Design review of the part shown in the three views and the two pictorial views. Dimensions are in mm from the part's minimum x, y and z. A direction names the side the tool comes from. Round coordinates to 2 decimals unless told otherwise and drop trailing zeros. Loops run counter-clockwise (first coordinate to the right, second up) from the corner with the lowest first, then second, coordinate; pieces in that order, holes last. Notation, with made-up numbers: (-27, 79) -> (11, 79) arc R11 cw to (11, 100) -> close; hole circle Ø6 at (68, 50). An arc over 180 degrees is marked (long way). Use CSV: the item, a comma, the result in double quotes. Start each with the question number.
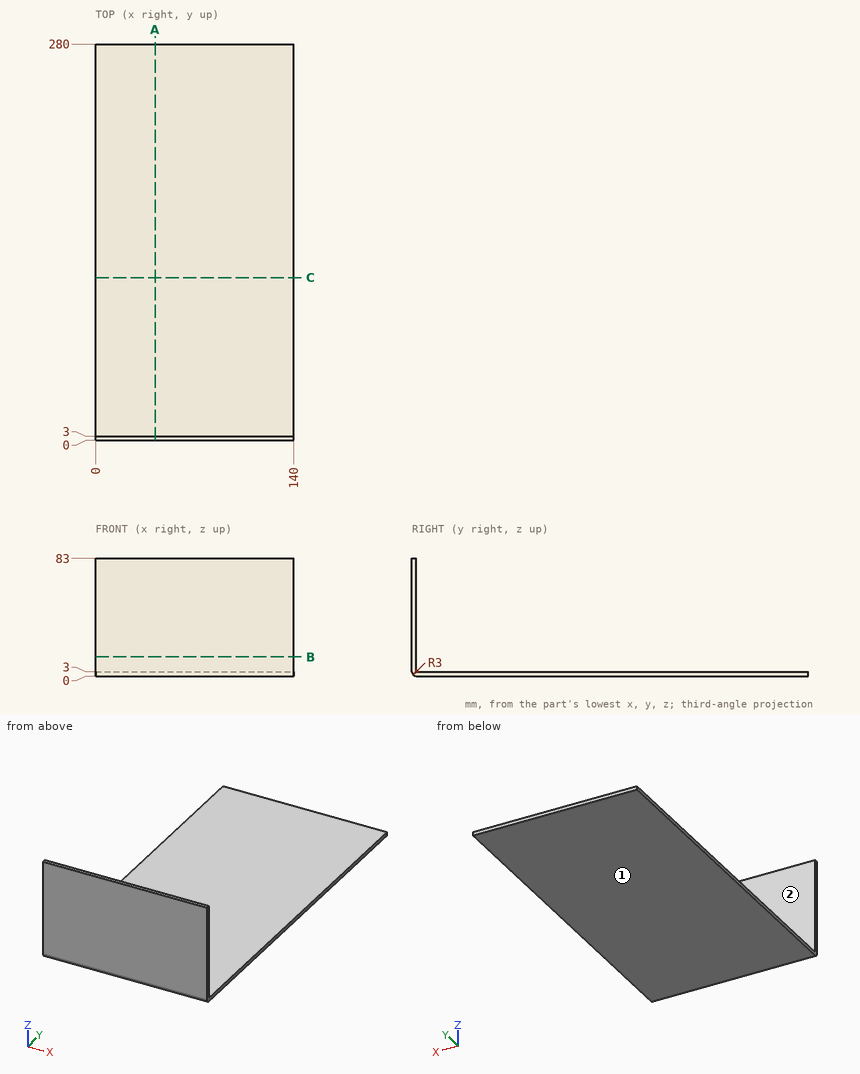
1. For the marked faces 1 and 2, list the 3-axis set-ups (+Z, -Z, +X, -X, +Y, -Y) from which the entire face can be reached by the end or side of a thin tool; tool diameter is ignored.
2. For line 1 along Z through (x, y) = (46.5, 228), list the stretches that pass through material, from the lowest coordinate up. Write a range as from..to.
3. Take a section at A-A, the plane x = 42. Give the boundary of the cut face in (y, z), then the cut area to 3 significant figures.
4. Take a section at B-B, the plane z = 13.5. Give the boundary of the cut face in (x, y).
5. Clearance check with flat-ended pins moving along their axes: P1, Ø4, axis at x = 54, z = 54, coming from the +Y side; P2, Ø8, axis at x = 93.5, y = 219, coming from the +Z side. State where each tip first meets the part, or that it passes through.
Results:
1,face 1,"-Z, +X, -X, +Y, -Y"
1,face 2,"+Z, +X, -X, +Y"
2,line 1,"0..3"
3,outline,"(0, 3) arc R3 ccw to (3, 0) -> (280, 0) -> (280, 3) -> (3, 3) -> (3, 83) -> (0, 83) -> close"
3,area,"1,080 mm²"
4,outline,"(0, 0) -> (140, 0) -> (140, 3) -> (0, 3) -> close"
5,P1,"y = 3"
5,P2,"z = 3"
